```python
from build123d import *

# Parameters (mm, degrees)
BOSS_EXTRUDE1_DEPTH = 880


with BuildPart() as part:
    # Sketch1 → Boss-Extrude1 (new body)
    with BuildSketch(Plane(origin=(0, 0, 0), x_dir=(1, 0, 0), z_dir=(0, 1, 0))):
        with BuildLine():
            Line((-20, -30), (20, -30))
            ThreePointArc((20, -30), (27.071067812, -27.071067812), (30, -20))
            Line((30, -20), (30, 20))
            ThreePointArc((30, 20), (27.071067812, 27.071067812), (20, 30))
            Line((20, 30), (-20, 30))
            ThreePointArc((-20, 30), (-27.071067812, 27.071067812), (-30, 20))
            Line((-30, 20), (-30, -20))
            ThreePointArc((-30, -20), (-27.071067812, -27.071067812), (-20, -30))
        make_face()
        with BuildLine():
            Line((-26, -20), (-26, 20))
            ThreePointArc((-26, 20), (-24.242640687, 24.242640687), (-20, 26))
            Line((-20, 26), (20, 26))
            ThreePointArc((20, 26), (24.242640687, 24.242640687), (26, 20))
            Line((26, 20), (26, -20))
            ThreePointArc((26, -20), (24.242640687, -24.242640687), (20, -26))
            Line((20, -26), (-20, -26))
            ThreePointArc((-20, -26), (-24.242640687, -24.242640687), (-26, -20))
        make_face(mode=Mode.SUBTRACT)
    extrude(amount=BOSS_EXTRUDE1_DEPTH)


solid = part.part
```
The model under review builds one solid part; all positions refer to its coordinate system, in mm. A direction names the side the tool comes from. Round coordinates to 2 decimals unless told otherwise and drop trailing zeros. Loops run counter-clockwise (first coordinate to the right, second up) from the corner with the lowest first, then second, coordinate; pieces in that order, holes last. Notation, with made-up numbers: M 10.25,30 L 15.25,30 A15 cw 15.25,47 Z; hole C 39,74 d7. An arc over 180 degrees is marked long. Put each result on its own line as item: value.
Q1. Consider section C-C, the plane y = 66. Give the boundary of the cut face in (x, z), then the cut area to 3 significant figures.
Result set:
outline: M -30,-20 A10 ccw -20,-30 L 20,-30 A10 ccw 30,-20 L 30,20 A10 ccw 20,30 L -20,30 A10 ccw -30,20 Z; hole M -26,-20 A6 ccw -20,-26 L 20,-26 A6 ccw 26,-20 L 26,20 A6 ccw 20,26 L -20,26 A6 ccw -26,20 Z
area: 841 mm²
Q2. Mouldability with a two-part tool opening along Z and no side actions: class faces 3 (the flat face through (0, 434, 30)), 4 (the flat face through (0, 434, -30)), 5 (the flat face through (26, 434, 0)) as released by +Z, released by -Z, zero draft, split by the parting line, or undercut.
Result set:
face 3: released by +Z
face 4: released by -Z
face 5: undercut
Q3. Machinability: for faces 1 (the flat face through (-30, 434, 0)), 2 (the flat face through (-26, 434, 0)), which of the approach directions +Z, -Z, +X, -X, +Y, -Y give a long, thin tool a straight path to every point of the face, cutting with its end or side? Answer none if there is none.
Result set:
face 1: +Z, -Z, -X, +Y, -Y
face 2: +Y, -Y
Q4. To check wall thickness, follow L1, parallel to X at y = 95, z = -20; L2, parallel to X at y = 610, z = -21. State the ranges of each line that lie inside material, in increasing order.
Result set:
L1: x = -30 to -26, 26 to 30
L2: x = -29.95 to -25.92, 25.92 to 29.95
Q5. Consider section B-B, the plane z = -10. Give the boundary of the cut face in (x, y), then the cut area to 3 significant figures.
Result set:
outline: M -30,0 L -26,0 L -26,880 L -30,880 Z; M 26,0 L 30,0 L 30,880 L 26,880 Z
area: 7,040 mm²
Q6. Consider section A-A, the plane x = -2. Give the boundary of the cut face in (y, z).
Result set:
outline: M 0,-30 L 880,-30 L 880,-26 L 0,-26 Z; M 0,26 L 880,26 L 880,30 L 0,30 Z
